Source: CAD feature listing. Evaluate the final solid. Frame: model axes, mm. A direction names the side the tool comes from. Round coordinates to 2 decimals unless told otherwise and drop trailing zeros. Loops run counter-clockwise (first coordinate to the right, second up) from the corner with the lowest first, then second, coordinate; pieces in that order, holes last. Notation, with made-up numbers: M 45,87.25 L 99,87.25 A25 ccw 99,118.25 Z; hole C 12.25,-12 d11. An arc over 180 degrees is marked long. Write each question's results on one line, items separated by ' | '. Start each with the question number.
1. Set-up query: faces 1 (the flat face through (-5, -5, -31.04)), 2 (the cylindrical face through (10, 3.2, 33)), 3 (the flat face through (8, 12, -27)), 4 (the flat face through (0, 10.92, 18)). Return all of +Z, -Z, +X, -X, +Y, -Y with unobstructed straight access to the full face (end or side cutting, diameter ignored); none if empty.
2. Draft query along Y for faces 5 (the flat face through (0, 10.92, -18)), 6 (the flat face through (5, -5, 31.04)), 7 (the cylindrical face through (10, 3.2, -33)), 8 (the cylindrical face through (0.108, 15.129, 15.544)). Return one class per face: released by +Y, released by -Y, zero draft, split by the parting line, or undercut.
3. Section A-A on x = 0. Give the number of separate pieces and of enclosed holes in the cut face, and give its area (3 significant figures).
4. Ray query, line 1 (Y direction, x = 11.7, z = -25); line 2 (Y direction, x = -3.25, z = 24.5); line 3 (X direction, y = 13.5, z = 18). Return the intervals inside material, ascending.
5. Section C-C on z = 25. Output: boundary loops of the cut face in (x, y), and give its area (3 significant figures).
6. Contact query for flat-ended pins moving along their axis: pin 1 Ø5.5 at (y, z) = (14, -25) entering from +X; pin 2 Ø1.5 at (x, y) = (-2.5, 5) entering from +Z; pin 3 Ø2.5 at (x, z) = (0.5, 17.5) entering from +Y. Output: stop coordinate, or through.
7. Section D-D on y = -4. Output: boundary loops of the cut face in (x, z).
from build123d import *

# Parameters (mm, degrees)
EXTRUDE_1_DEPTH          = 14
EXTRUDE_1_DEPTH_BACK     = 14
SKETCH_3_W               = 6
SKETCH_3_H               = 4
SKETCH_4_W               = 6
SKETCH_4_H               = 4
CUT_EXTRUDE_1_DEPTH      = 35
CUT_EXTRUDE_1_DEPTH_BACK = 35
SKETCH_9_W               = 32
SKETCH_9_H               = 38
CUT_EXTRUDE_2_DEPTH      = 34
CUT_EXTRUDE_2_DEPTH_BACK = 34
SKETCH_10_W              = 32
SKETCH_10_H              = 74


with BuildPart() as part:
    # 草图1 → 凸台-拉伸1 (new, two sides: drawn at the far end of the back side and taken through both)
    with BuildSketch(Plane(origin=(0, 0, 0), x_dir=(0, 0, -1), z_dir=(1, 0, 0)).offset(-EXTRUDE_1_DEPTH_BACK)):
        Polygon((-35, -13.5), (-34.5, -14), (34.5, -14), (35, -13.5), (35, 19.5), (34.5, 20), (-34.5, 20), (-35, 19.5), align=None)
    extrude(amount=EXTRUDE_1_DEPTH + EXTRUDE_1_DEPTH_BACK)

    # 草图2 → 切除-旋转1 (revolve, cut)
    with BuildSketch(Plane(origin=(0, 0, 0), x_dir=(0, 0, -1), z_dir=(1, 0, 0)), mode=Mode.PRIVATE) as cut_revolve_1_sk:
        Polygon((-35, 0), (-35, 10.5), (-31.04, 10.5), (-31.04, 6), (31.04, 6), (31.04, 10.5), (35, 10.5), (35, 0), align=None)
    revolve(cut_revolve_1_sk.sketch.rotate(Axis((0, 0, -35), (0, 0, 1)), 270), axis=Axis((0, 0, -35), (0, 0, 1)), mode=Mode.SUBTRACT)

    # 草图3 → 切除-旋转2 (revolve, cut)
    with BuildSketch(Plane.XY.offset(25), mode=Mode.PRIVATE) as cut_revolve_2_sk:
        with Locations((11, 16)):
            Rectangle(SKETCH_3_W, SKETCH_3_H)
    revolve(cut_revolve_2_sk.sketch.rotate(Axis((14, 14, 25), (-1, 0, 0)), 270), axis=Axis((14, 14, 25), (-1, 0, 0)), mode=Mode.SUBTRACT)

    # 草图4 → 切除-旋转3 (revolve, cut)
    with BuildSketch(Plane.XY.offset(-25), mode=Mode.PRIVATE) as cut_revolve_3_sk:
        with Locations((11, 16)):
            Rectangle(SKETCH_4_W, SKETCH_4_H)
    revolve(cut_revolve_3_sk.sketch.rotate(Axis((14, 14, -25), (-1, 0, 0)), 270), axis=Axis((14, 14, -25), (-1, 0, 0)), mode=Mode.SUBTRACT)

    # 草图5 → 切除-旋转4 (revolve, cut)
    with BuildSketch(Plane(origin=(0, 0, 0), x_dir=(0, 0, -1), z_dir=(1, 0, 0)), mode=Mode.PRIVATE) as cut_revolve_4_sk:
        Polygon((18, 20), (21, 20), (20.4585, 19.4585), (20.4585, 10.92), (18, 10.92), align=None)
    revolve(cut_revolve_4_sk.sketch.rotate(Axis((0, 10.92, -18), (0, 1, 0)), 180), axis=Axis((0, 10.92, -18), (0, 1, 0)), mode=Mode.SUBTRACT)

    # 草图6 → 切除-旋转5 (revolve, cut)
    with BuildSketch(Plane(origin=(0, 0, 0), x_dir=(0, 0, -1), z_dir=(1, 0, 0)), mode=Mode.PRIVATE) as cut_revolve_5_sk:
        Polygon((-18, 20), (-15, 20), (-15.5415, 19.4585), (-15.5415, 10.92), (-18, 10.92), align=None)
    revolve(cut_revolve_5_sk.sketch.rotate(Axis((0, 10.92, 18), (0, 1, 0)), 180), axis=Axis((0, 10.92, 18), (0, 1, 0)), mode=Mode.SUBTRACT)

    # 草图7 → 切除-旋转6 (revolve, cut)
    with BuildSketch(Plane.XY.offset(-25), mode=Mode.PRIVATE) as cut_revolve_6_sk:
        Polygon((-14, 14), (-14, 16.5), (-13.567, 16.067), (8, 16.067), (8, 14), align=None)
    revolve(cut_revolve_6_sk.sketch.rotate(Axis((8, 14, -25), (-1, 0, 0)), 270), axis=Axis((8, 14, -25), (-1, 0, 0)), mode=Mode.SUBTRACT)

    # 草图8 → 切除-旋转7 (revolve, cut)
    with BuildSketch(Plane.XY.offset(25), mode=Mode.PRIVATE) as cut_revolve_7_sk:
        Polygon((-14, 14), (-14, 16.5), (-13.567, 16.067), (8, 16.067), (8, 14), align=None)
    revolve(cut_revolve_7_sk.sketch.rotate(Axis((8, 14, 25), (-1, 0, 0)), 270), axis=Axis((8, 14, 25), (-1, 0, 0)), mode=Mode.SUBTRACT)

    # 草图9 → 切除-拉伸1 (cut, two sides: drawn at the far end of the back side and taken through both)
    with BuildSketch(Plane.XY.offset(-CUT_EXTRUDE_1_DEPTH_BACK)):
        with Locations((0, 3)):
            Rectangle(SKETCH_9_W, SKETCH_9_H)
        Polygon((-14, -13.5), (-13.5, -14), (13.5, -14), (14, -13.5), (14, 19.5), (13.5, 20), (-13.5, 20), (-14, 19.5), align=None, mode=Mode.SUBTRACT)
    extrude(amount=CUT_EXTRUDE_1_DEPTH + CUT_EXTRUDE_1_DEPTH_BACK, mode=Mode.SUBTRACT)

    # 草图10 → 切除-拉伸2 (cut, two sides: drawn at the far end of the back side and taken through both)
    with BuildSketch(Plane(origin=(0, 0, 0), x_dir=(1, 0, 0), z_dir=(0, 1, 0)).offset(-CUT_EXTRUDE_2_DEPTH_BACK)):
        Rectangle(SKETCH_10_W, SKETCH_10_H)
        Polygon((-14, -34.5), (-13.5, -35), (13.5, -35), (14, -34.5), (14, 34.5), (13.5, 35), (-13.5, 35), (-14, 34.5), align=None, mode=Mode.SUBTRACT)
    extrude(amount=CUT_EXTRUDE_2_DEPTH + CUT_EXTRUDE_2_DEPTH_BACK, mode=Mode.SUBTRACT)


solid = part.part
Taken from the geometry:
1) face 1: -Z | face 2: +Z | face 3: +X | face 4: +Y
2) face 5: released by +Y | face 6: undercut | face 7: undercut | face 8: zero draft
3) separate pieces: 2 | enclosed holes: 2 | area: 1,350 mm^2
4) line 1: -14 to 10, 18 to 20 | line 2: -14 to -5.04, 5.04 to 11.99, 16.01 to 20 | line 3: -14 to -2.46, 2.46 to 14
5) outline: M -14,-13.5 L -13.5,-14 L 13.5,-14 L 14,-13.5 L 14,10 L 8,10 L 8,11.93 L -13.57,11.93 L -14,11.5 Z; M -14,16.5 L -13.57,16.07 L 8,16.07 L 8,18 L 14,18 L 14,19.5 L 13.5,20 L -13.5,20 L -14,19.5 Z; hole C 0,0 d12 | area: 699 mm^2
6) pin 1: x = 8 | pin 2: z = 31.04 | pin 3: y = 10.92
7) outline: M -14,-34.5 L -13.5,-35 L -9.71,-35 L -9.71,-31.04 L -4.47,-31.04 L -4.47,31.04 L -9.71,31.04 L -9.71,35 L -13.5,35 L -14,34.5 Z; M 4.47,-31.04 L 9.71,-31.04 L 9.71,-35 L 13.5,-35 L 14,-34.5 L 14,34.5 L 13.5,35 L 9.71,35 L 9.71,31.04 L 4.47,31.04 Z
